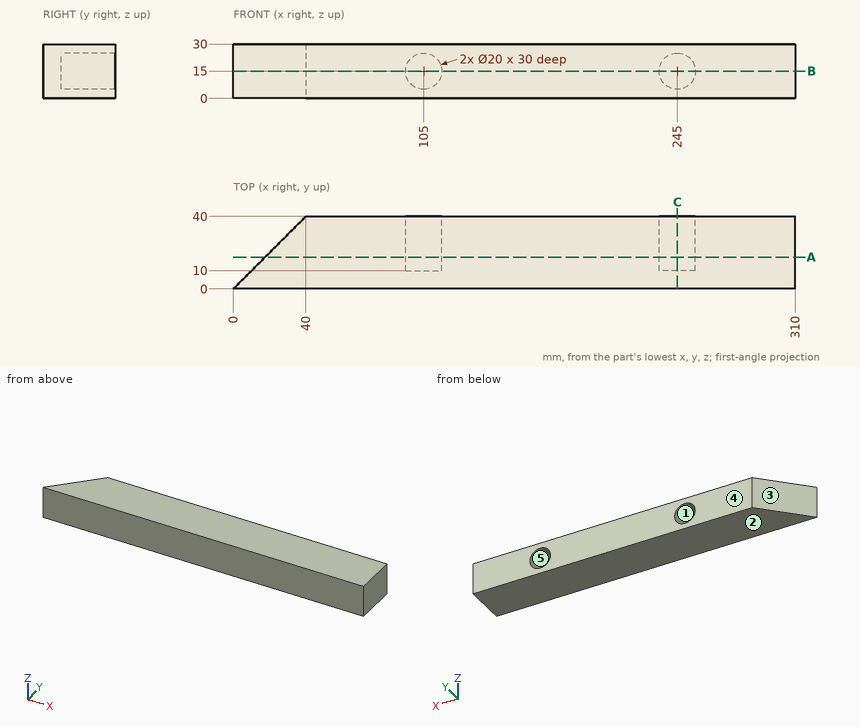
Job drawing, mm, ordinate dimensions from the low corner. One solid piece. A direction names the side the tool comes from. Give positions to 0.01 mm unless a question says otherwise; leave off trailing zeros. Loops run counter-clockwise (first coordinate to the right, second up) from the corner with the lowest first, then second, coordinate; pieces in that order, holes last. Notation, with made-up numbers: (-39.75, 36.25) -> (8.25, 36.25) arc R27 ccw to (8.25, 58.25) -> close; hole circle Ø6 at (56, 64.25). An arc over 180 degrees is marked (long way). Write each question's results on one line, items separated by ' | '.
(1) Cut at B-B on z = 15. List the corners of the cut face in (x, y).
Geometry results:
outline: (0, 0) -> (310, 0) -> (310, 40) -> (255, 40) -> (255, 10) -> (235, 10) -> (235, 40) -> (115, 40) -> (115, 10) -> (95, 10) -> (95, 40) -> (40, 40) -> close
(2) Cut at A-A on y = 17.5. List the corners of the cut face in (x, z).
Geometry results:
outline: (17.5, 0) -> (310, 0) -> (310, 30) -> (17.5, 30) -> close; hole circle Ø20 at (105, 15); hole circle Ø20 at (245, 15)
(3) Flat gauge pins, fed straight in: pin 1 Ø4 at (y, z) = (24.5, 21) entering from -X; pin 2 Ø1 at (y, z) = (23.5, 15.5) entering from -X; pin 3 Ø12 at (x, z) = (105, 15) entering from +Y. Where does each tip first touch, or does it go through?
Geometry results:
pin 1: stops at x = 22.5 | pin 2: stops at x = 23 | pin 3: stops at y = 10
(4) Tool access for the marked faces 4 and 5: list every direction of +Z, -Z, +X, -X, +Y, -Y with a clear straight run to the whole face (end or side of a thin tool).
Geometry results:
face 4: +Z, -Z, +X, -X, +Y | face 5: +Y
(5) Pull direction Z, two halves, no side cores. Call the marked faces 1, 2 and 3: released by +Z, released by -Z, zero draft, split by the parting line, or undercut.
Geometry results:
face 1: undercut | face 2: released by -Z | face 3: zero draft
(6) Probe line 1 along X through (y, z) = (18.75, 15); line 2 along Z through (x, y) = (105, 17); line 3 along X through (y, z) = (22.25, 15). List the from-to ranges inside material, lowest first.
Geometry results:
line 1: x = 18.75 to 95, 115 to 235, 255 to 310 | line 2: z = 0 to 5, 25 to 30 | line 3: x = 22.25 to 95, 115 to 235, 255 to 310
(7) Cut at C-C on x = 245. List the corners of the cut face in (y, z), and give its area (3 significant figures).
Geometry results:
outline: (0, 0) -> (40, 0) -> (40, 5) -> (10, 5) -> (10, 25) -> (40, 25) -> (40, 30) -> (0, 30) -> close | area: 600 mm²
